```python
from build123d import *

# Parameters (mm, degrees)
SKETCH_11_R         = 2
EXTRUDE_3_DEPTH     = 100
SKETCH_20_R         = 4
EXTRUDE_4_DEPTH     = 10
SKETCH_16_W         = 2.1
SKETCH_16_H         = 5
CUT_EXTRUDE_5_DEPTH = 200
SKETCH_18_R         = 1
CUT_EXTRUDE_7_DEPTH = 200
SKETCH_19_R         = 1
CUT_EXTRUDE_8_DEPTH = 5
FILLET_1_R          = 0.2
FILLET_2_R          = 0.2


with BuildPart() as part:
    # 草图11 → 凸台-拉伸3 (new body)
    with BuildSketch(Plane.XZ):
        with Locations(Location((0, 0, 0), (0, 0, 270))):
            Circle(SKETCH_11_R)
    extrude(amount=EXTRUDE_3_DEPTH)

    # 草图20 → 凸台-拉伸4 (add)
    with BuildSketch(Plane.XZ.offset(100)):
        with Locations(Location((0, 0, 0), (0, 0, 270))):
            Circle(SKETCH_20_R)
    extrude(amount=-EXTRUDE_4_DEPTH)

    # 草图16 → 切除-拉伸5 (cut, symmetric)
    with BuildSketch(Plane.XY):
        with Locations((0, -97.5)):
            Rectangle(SKETCH_16_W, SKETCH_16_H)
    extrude(amount=CUT_EXTRUDE_5_DEPTH, both=True, mode=Mode.SUBTRACT)

    # 草图18 → 切除-拉伸7 (cut, symmetric)
    with BuildSketch(Plane(origin=(-1.05, 0, 0), x_dir=(0, 0, -1), z_dir=(1, 0, 0))):
        with Locations(Location((0, -97.8, 0), (0, 0, 90))):
            Circle(SKETCH_18_R)
    extrude(amount=CUT_EXTRUDE_7_DEPTH, both=True, mode=Mode.SUBTRACT)

    # 草图19 → 切除-拉伸8 (cut, symmetric)
    with BuildSketch(Plane(origin=(0, 0, 0), x_dir=(0, 0, -1), z_dir=(1, 0, 0))):
        with Locations((0, -3)):
            Circle(SKETCH_19_R)
    extrude(amount=CUT_EXTRUDE_8_DEPTH, both=True, mode=Mode.SUBTRACT)

    # 圆角1
    fillet_1_edges = [part.edges().sort_by_distance(p)[0] for p in [
        (-4, -100, 0),
        (1.05, -100, 0),
        (-1.05, -100, 0),
        (4, -100, 0),
    ]]
    fillet(fillet_1_edges, radius=FILLET_1_R)

    # 圆角2
    fillet_2_edges = [part.edges().sort_by_distance(p)[0] for p in [
        (-1.05, -95, 0),
        (1.05, -95, 0),
    ]]
    fillet(fillet_2_edges, radius=FILLET_2_R)


solid = part.part
```
Here's how the part is built. I have some questions about the finished solid (model axes, mm). A direction names the side the tool comes from. Give positions to 0.01 mm unless a question says otherwise; leave off trailing zeros. Loops run counter-clockwise (first coordinate to the right, second up) from the corner with the lowest first, then second, coordinate; pieces in that order, holes last. Notation, with made-up numbers: (15.25, -24.75) -> (57.25, -24.75) arc R31 ccw to (57.25, 12.25) -> close; hole circle Ø7 at (-25.5, -30). An arc over 180 degrees is marked (long way). Use one line per item in the form item = value. Start each with the question number.
1) Imagine slicing it at B-B (x = 0). Please give me the cut outline in (y, z), then the cut area to 3 significant figures.
2) Which directions (+Z, -Z, +X, -X, +Y, -Y) give clear straight access to the entire face, cutting with the end or side of a thin tool? Please do faces 4 (the face through (-1.05, -97, 1)), 5 (the face through (-2, -44, 0)), 6 (the face through (-2, -100, 0)).
3) Imagine slicing it at C-C (y = -97.8). Please give me the cut outline in (x, z), then the cut area to 3 significant figures.
4) Imagine slicing it at A-A (z = 0). Count the separate pieces of the cut face and the enclosed holes in it, then the cut area to 3 significant figures.
5) Please list where these lines run through material, in increasing order: line 1 along Y through (x, z) = (2.5, 0); line 2 along Y through (x, z) = (-0.65, 0); line 3 along Z through (x, y) = (-0.25, -3).
6) Imagine slicing it at D-D (y = -64). Please give me the cut outline in (x, z), then the cut area to 3 significant figures.
7) Thinking about a two-plate mould opening in Y: for faces 1 (the face through (2, -100, 0)), 2 (the face through (1.05, -97, 1)), 3 (the face through (2.547, -96.876, -0.383)), which applies, +Y half, -Y half, draft (parallel to the pull), parting line (faces both ways), or undercut?
8) For P1, Ø2.5, axis at y = -97.8, z = 0, coming from the -X side; P2, Ø2, axis at y = -70.5, z = 0, coming from the +X side; P3, Ø3, axis at y = -3, z = 0, coming from the -X side; P4, Ø0.5, axis at x = -0.5, z = -1, coming from the -Y side, each with a flat end and sliding along its axis, tell me the tip position at first contact or that it passes through.
Check values:
q1.outline = (-95, -4) -> (-90, -4) -> (-90, -2) -> (0, -2) -> (0, 2) -> (-90, 2) -> (-90, 4) -> (-95, 4) -> close; hole circle Ø2 at (-3, 0)
q1.area = 397 mm^2
q2.face_4 = +Z, -Z, -Y
q2.face_5 = +Y
q2.face_6 = +Z, -Z, +X, -X, -Y
q3.outline = (-3.87, -1) arc R4 ccw to (-1.05, -3.86) -> (-1.05, -1) -> close; (-3.87, 1) -> (-1.05, 1) -> (-1.05, 3.86) arc R4 ccw to start; (1.05, -3.86) arc R4 ccw to (3.87, -1) -> (1.05, -1) -> close; (1.05, 1) -> (3.87, 1) arc R4 ccw to (1.05, 3.86) -> close
q3.area = 22.0 mm^2
q4.separate_pieces = 4
q4.enclosed_holes = 0
q4.area = 410 mm^2
q5.line_1 = -100 to -98.8, -96.8 to -90
q5.line_2 = -95 to -4, -2 to 0
q5.line_3 = -1.98 to -1, 1 to 1.98
q6.outline = circle Ø4 at (0, 0)
q6.area = 12.6 mm^2
q7.face_1 = -Y half
q7.face_2 = draft
q7.face_3 = undercut
q8.P1 = -4
q8.P2 = 2
q8.P3 = -2
q8.P4 = -95
